from build123d import *

# Parameters (mm, degrees)
SKETCH1_R                = 175
BOSS_EXTRUDE2_DEPTH      = 150
SHELL2_T                 = -5
SKETCH2_R                = 60
BOSS_EXTRUDE3_DEPTH      = 50
SKETCH_3_3_R             = 15
CUT_EXTRUDE1_DEPTH       = 50
BOSS_EXTRUDE5_DEPTH      = 50
BOSS_EXTRUDE5_DEPTH_BACK = 20
SKETCH_3_3_2_R           = 18
SKETCH_3_3_2_R_2         = 15
SKETCH5_R                = 8
BOSS_EXTRUDE6_DEPTH      = 40
BOSS_EXTRUDE7_START      = -5
SKETCH6_R                = 170
SKETCH6_R_2              = 160
BOSS_EXTRUDE7_DEPTH      = 5
SKETCH7_R                = 2.5
CUT_EXTRUDE2_DEPTH       = 10


with BuildPart() as part:
    # Sketch1 → Boss-Extrude2 (new body)
    with BuildSketch(Plane(origin=(0, 0, 0), x_dir=(1, 0, 0), z_dir=(0, 1, 0))):
        with Locations(Location((0, 0, 0), (0, 0, 270))):
            Circle(SKETCH1_R)
    extrude(amount=BOSS_EXTRUDE2_DEPTH)

    # Shell2
    shell2_openings = [part.faces().sort_by_distance(p)[0] for p in [
        (0, 150, 0),
    ]]
    offset(amount=SHELL2_T, openings=shell2_openings, kind=Kind.INTERSECTION)

    # Sketch2 → Boss-Extrude3 (add)
    with BuildSketch(Plane(origin=(0, 5, 0), x_dir=(1, 0, 0), z_dir=(0, 1, 0))):
        with Locations(Location((0, 0, 0), (0, 0, 270))):
            Circle(SKETCH2_R)
    extrude(amount=BOSS_EXTRUDE3_DEPTH)

    # Sketch 3_3 → Cut-Extrude1 (cut)
    with BuildSketch(Plane.ZY.offset(175)):
        with Locations((0, 96.363123984)):
            Circle(SKETCH_3_3_R)
    extrude(amount=-CUT_EXTRUDE1_DEPTH, mode=Mode.SUBTRACT)

    # Sketch 3_3 2 → Boss-Extrude5 (add, two sides: drawn at the far end of the back side and taken through both)
    with BuildSketch(Plane.ZY.offset(175).offset(-BOSS_EXTRUDE5_DEPTH_BACK)):
        with Locations((0, 96.363123984)):
            Circle(SKETCH_3_3_2_R)
        with Locations((0, 96.363123984)):
            Circle(SKETCH_3_3_2_R_2, mode=Mode.SUBTRACT)
    extrude(amount=BOSS_EXTRUDE5_DEPTH + BOSS_EXTRUDE5_DEPTH_BACK)

    # Sketch5 → Boss-Extrude6 (add)
    with BuildSketch(Plane(origin=(0, 55, 0), x_dir=(1, 0, 0), z_dir=(0, 1, 0))):
        with Locations(Location((0, 0, 0), (0, 0, 270))):
            Circle(SKETCH5_R)
    extrude(amount=BOSS_EXTRUDE6_DEPTH)

    # Sketch6 → Boss-Extrude7 (add)
    with BuildSketch(Plane(origin=(0, 150, 0), x_dir=(1, 0, 0), z_dir=(0, 1, 0)).offset(BOSS_EXTRUDE7_START)):
        with Locations(Location((0, 0, 0), (0, 0, 270))):
            Circle(SKETCH6_R)
        with Locations(Location((0, 0, 0), (0, 0, 270))):
            Circle(SKETCH6_R_2, mode=Mode.SUBTRACT)
    extrude(amount=BOSS_EXTRUDE7_DEPTH)

    # Sketch7 → Cut-Extrude2 (cut)
    with BuildSketch(Plane(origin=(0, 150, 0), x_dir=(1, 0, 0), z_dir=(0, 1, 0))):
        with Locations(Location((0, -170, 0), (0, 0, 270))):
            Circle(SKETCH7_R)
        with Locations(Location((-170, 0, 0), (0, 0, 270))):
            Circle(SKETCH7_R)
        with Locations(Location((0, 170, 0), (0, 0, 270))):
            Circle(SKETCH7_R)
        with Locations(Location((170, 0, 0), (0, 0, 270))):
            Circle(SKETCH7_R)
    extrude(amount=-CUT_EXTRUDE2_DEPTH, mode=Mode.SUBTRACT)


solid = part.part
For this review, take the finished solid that the model builds, in its own axes (mm). A direction names the side the tool comes from. Give positions to 0.01 mm unless a question says otherwise; leave off trailing zeros. Loops run counter-clockwise (first coordinate to the right, second up) from the corner with the lowest first, then second, coordinate; pieces in that order, holes last. Notation, with made-up numbers: M -5.5,-26 L 8.5,-26 A18 ccw 8.5,-8 Z; hole C 3,-18 d9. An arc over 180 degrees is marked long. Answer as a JSON object with one key per item and string values. Group by question number.
Q1. Mouldability with a two-part tool opening along Y and no side actions: class faces 5 (the cylindrical face through (-199.18, 114.21, -2.34)), 6 (the cylindrical face through (-162.4, 101.77, 17.17)), 7 (the flat face through (-155, 110, -7)) as +Y half, -Y half, draft (parallel to the pull), parting line (faces both ways), or undercut.
Q2. For probe 1 along Y at (x, z) = (-159, 0); probe 2 along X at (y, z) = (147.1, 0); probe 3 along X at (y, z) = (144, 0), list the stretches that pass through material, from the lowest coordinate up. Write a range as [from, to].
Q3. Tool access review of faces 1 (the flat face through (0, 95, 0)), 2 (the flat face through (-73, 5, -2)), 3 (the cylindrical face through (-156.195, 147.465, -34.685)), 4 (the flat face through (2, 0, -2)): name each direction out of +Z, -Z, +X, -X, +Y, -Y from which nothing blocks a thin tool from reaching the whole face with its end or side.
Q4. Add section B-B on y = 14. Give the boundary of the cut face in (x, z).
Q5. Insertion check: P1, Ø0.8, axis at x = -171, z = 0, coming from the +Y side; P2, Ø8, axis at x = 32, y = 30, coming from the +Z side; P3, Ø4, axis at x = -87, z = 63.5, coming from the -Y side; P4, Ø2, axis at y = 46.5, z = 119, coming from the +X side. Each pin has a flat end and moves straight along its axis. Give the tip position at first contact, or say it passes through.
Q6. Add section D-D on x = 145.5. Give the boundary of the cut face in (y, z), and give its area (3 significant figures).
Q7. Add section A-A on y = 128. Give the boundary of the cut face in (x, z).
Q8. Add section C-C on z = 32.5. Give the boundary of the cut face in (x, y).
Checked values:
{
 "1": {"face 5": "parting line", "face 6": "undercut", "face 7": "draft"},
 "2": {"probe 1": "[0, 5], [78.36, 81.36], [111.36, 114.36]", "probe 2": "[-175, -172.5], [-167.5, -160], [160, 167.5], [172.5, 175]", "probe 3": "[-175, -172.5], [172.5, 175]"},
 "3": {"face 1": "-X, +Y", "face 2": "none", "face 3": "+Y", "face 4": "+Z, -Z, +X, -X, -Y"},
 "4": {"outline": "C 0,0 d350; C 0,0 d120; hole C 0,0 d340"},
 "5": {"P1": "y = 140", "P2": "z = 172.75", "P3": "y = 0", "P4": "x = 129.23"},
 "6": {"outline": "M 0,-97.24 L 150,-97.24 L 150,-66.56 L 145,-66.56 L 145,-87.92 L 5,-87.92 L 5,87.92 L 145,87.92 L 145,66.56 L 150,66.56 L 150,97.24 L 0,97.24 Z", "area": "3,890 mm²"},
 "7": {"outline": "C 0,0 d350; hole C 0,0 d340"},
 "8": {"outline": "M -171.96,0 L 171.96,0 L 171.96,150 L 156.66,150 L 156.66,145 L 166.86,145 L 166.86,5 L 50.44,5 L 50.44,55 L -50.44,55 L -50.44,5 L -166.86,5 L -166.86,145 L -156.66,145 L -156.66,150 L -171.96,150 Z"}
}
